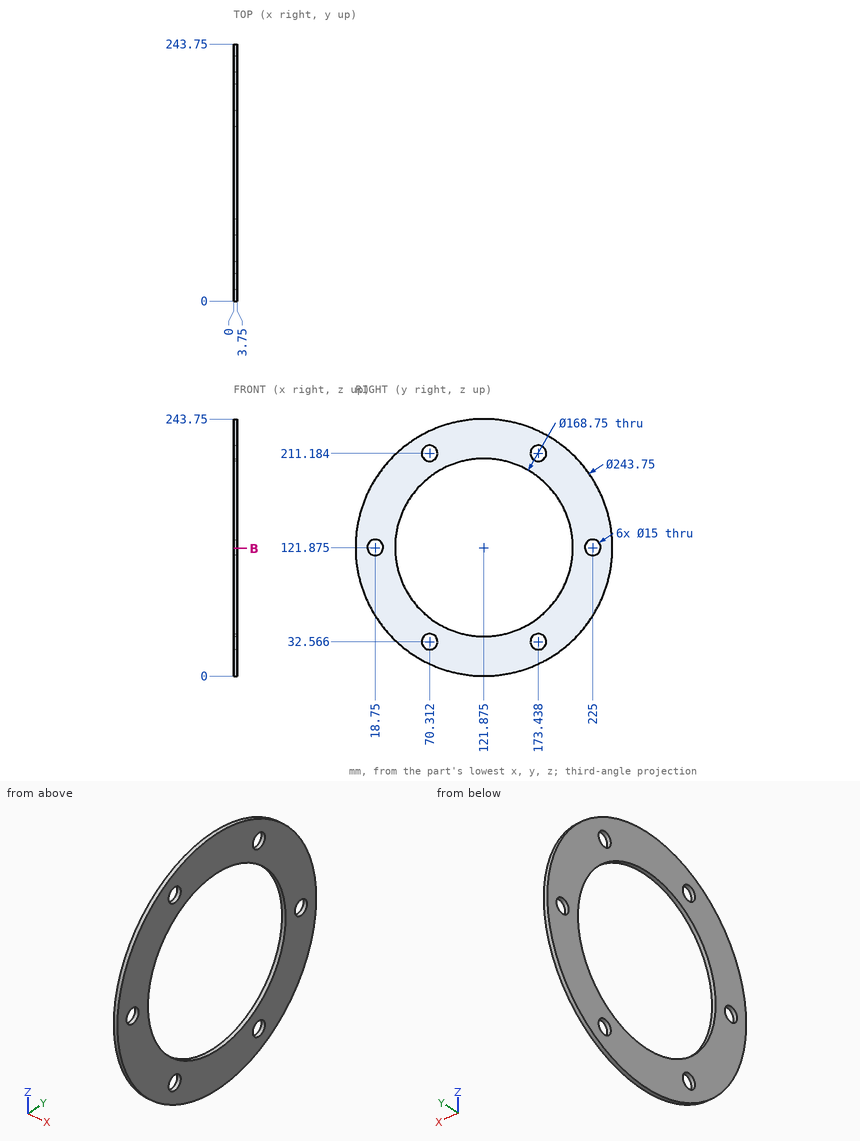
The figure shows three views and two pictorial views of one solid part (mm, origin at its lowest corner). Answer the questions. Round coordinates to 2 decimals unless told otherwise and drop trailing zeros. Write item = value, one per line. Start each with the question number.
1) Given pin 1 (24 mm diameter, centred on y = 173.44, z = 211.18, fed in from +X); pin 2 (1 mm diameter, centred on x = 2.5, z = 154, fed in from -Y) (1 decimal); pin 3 (9 mm diameter, centred on y = 18.75, z = 121.875, fed in from -X), each flat-ended and moving along its own axis, determine where each tip first touches the part or whether it passes through.
2) Straight lines are drawn through the part: L1, parallel to Z at x = 0.2, y = 177 (1 decimal); L2, parallel to Z at x = 0.9, y = 149; L3, parallel to Z at x = 2.75, y = 13 (1 decimal). For each, find the intervals that lie inside material, in ascending order.
3) Section B-B, the plane z = 121 is taken. Count the separate pieces of the cut face and the enclosed holes in it.
Results list:
q1.pin_1 = 3.75
q1.pin_2 = 4.2
q1.pin_3 = through
q2.L1 = 13.2 to 26, 39.2 to 58, 185.8 to 204.6, 217.8 to 230.6
q2.L2 = 3.06 to 41.98, 201.77 to 240.69
q2.L3 = 67.1 to 117.1, 126.7 to 176.6
q3.separate_pieces = 4
q3.enclosed_holes = 0
